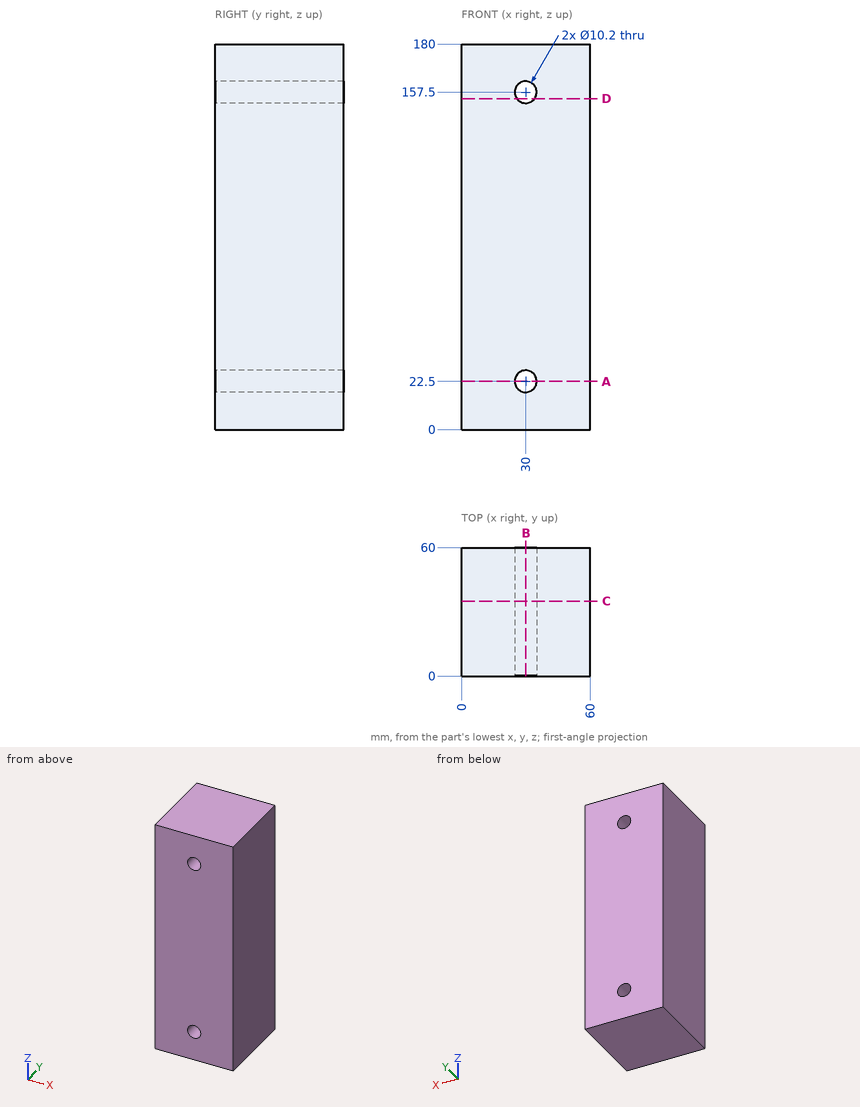
Check sheet for the drawn part. Datum: minimum x, y, z corner. Units: mm. Coordinates: 2 decimals unless noted, no trailing zeros. Order: outer loops, then holes, each group sorted by start corner. A loop starts at its lowest first (then second) coordinate and runs counter-clockwise, first axis right, second up. Notation, with made-up numbers: (0.25, 53) -> (8.25, 53) arc R29 cw to (8.25, 92) -> close; hole circle Ø9 at (6.5, 38.25). An arc over 180 degrees is marked (long way). Write each question's results on one line, items separated by ' | '. Start each with the question number.
1) Section check A-A (z = 22.5). Enter the section's corners in (x, y), and give its area (3 significant figures).
2) Section check B-B (x = 30). Enter the section's corners in (y, z).
3) Material ranges on line 1 along Z through (x, y) = (30, 30.5); line 2 along Z through (x, y) = (32, 17.5); line 3 along X through (y, z) = (36.5, 157.5), recorded low to high.
4) Section check D-D (z = 154.5). Enter the section's corners in (x, y).
5) Section check C-C (y = 35). Enter the section's corners in (x, z).
Checked values:
1) outline: (0, 0) -> (24.9, 0) -> (24.9, 60) -> (0, 60) -> close; (35.1, 0) -> (60, 0) -> (60, 60) -> (35.1, 60) -> close | area: 2,990 mm²
2) outline: (0, 0) -> (60, 0) -> (60, 17.4) -> (0, 17.4) -> close; (0, 27.6) -> (60, 27.6) -> (60, 152.4) -> (0, 152.4) -> close; (0, 162.6) -> (60, 162.6) -> (60, 180) -> (0, 180) -> close
3) line 1: 0 to 17.4, 27.6 to 152.4, 162.6 to 180 | line 2: 0 to 17.81, 27.19 to 152.81, 162.19 to 180 | line 3: 0 to 24.9, 35.1 to 60
4) outline: (0, 0) -> (25.88, 0) -> (25.88, 60) -> (0, 60) -> close; (34.12, 0) -> (60, 0) -> (60, 60) -> (34.12, 60) -> close
5) outline: (0, 0) -> (60, 0) -> (60, 180) -> (0, 180) -> close; hole circle Ø10.2 at (30, 22.5); hole circle Ø10.2 at (30, 157.5)
